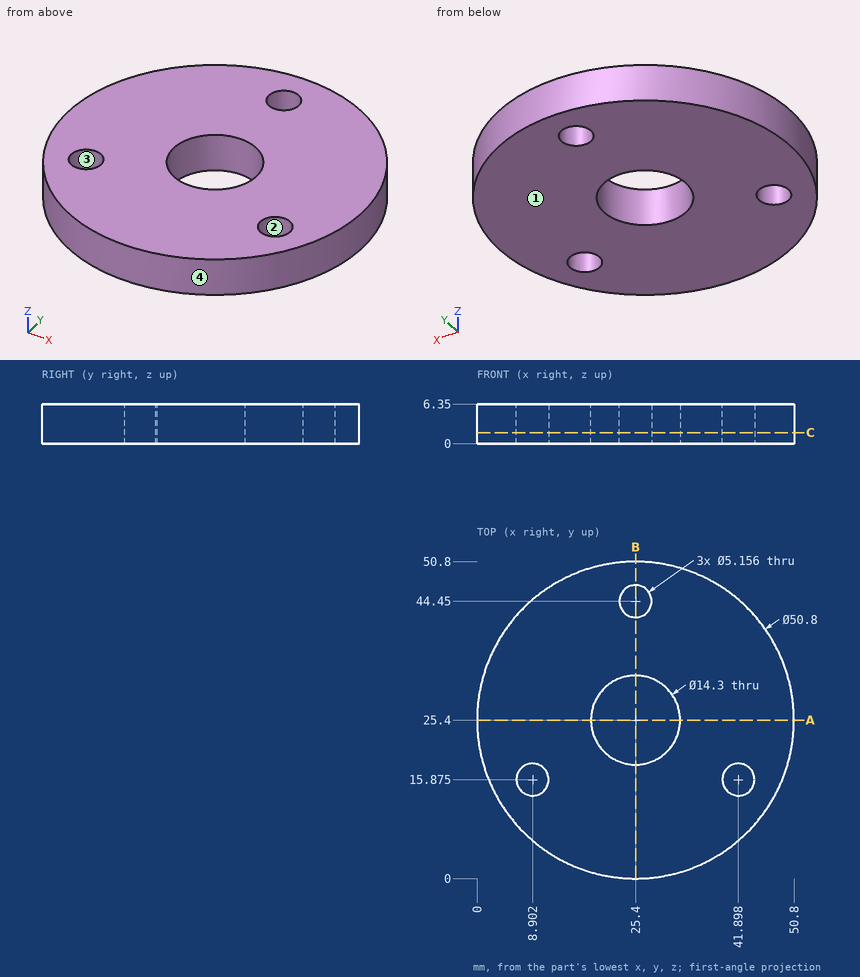
Answer from the drawing. Dimensions are ordinates in mm from the lowest x, y and z of the part. Give positions to 0.01 mm unless a question says otherwise; leave off trailing zeros. Order: outer loops, then holes, each group sorted by start corner. A loop starts at its lowest first (then second) coordinate and runs counter-clockwise, first axis right, second up.
(1) Find section B-B (x = 25.4). Give the vertices of the cut face in (y, z).
(2) Straight lines are drawn through the part: L1, parallel to Y at x = 25.4, z = 2.75; L2, parallel to X at y = 27, z = 2.25; L3, parallel to X at y = 20, z = 1. For each, find the intervals that lie inside material, in ascending order.
(3) Find section A-A (y = 25.4). Give the vertices of the cut face in (x, z), plus the area to 3 significant figures.
(4) Find section C-C (z = 1.75). Give the number of separate pieces and of enclosed holes in the cut face, plus the area to 3 significant figures.
(5) For a pull along X with two mould halves and no side action, classify the marked faces 1, 2, 3 and 4 as released by +X, released by -X, zero draft, split by the parting line, or undercut.
(6) Given pin 1 (1 mm diameter, centred on y = 33, z = 4, fed in from +X); pin 2 (18.5 mm diameter, centred on x = 25.4, y = 25.4, fed in from +Z); pin 3 (2 mm diameter, centred on x = 39, z = 1.5, fed in from -Y) (1 decimal), each flat-ended and moving along its own axis, determine where each tip first touches the part or whether it passes through.
Result sheet:
1. outline: (0, 0) - (18.25, 0) - (18.25, 6.35) - (0, 6.35) - close; (32.55, 0) - (41.87, 0) - (41.87, 6.35) - (32.55, 6.35) - close; (47.03, 0) - (50.8, 0) - (50.8, 6.35) - (47.03, 6.35) - close
2. L1: y = 0 to 18.25, 32.55 to 41.87, 47.03 to 50.8
2. L2: x = 0.05 to 18.43, 32.37 to 50.75
2. L3: x = 0.58 to 20.71, 30.09 to 50.22
3. outline: (0, 0) - (18.25, 0) - (18.25, 6.35) - (0, 6.35) - close; (32.55, 0) - (50.8, 0) - (50.8, 6.35) - (32.55, 6.35) - close
3. area: 232 mm2
4. separate pieces: 1
4. enclosed holes: 4
4. area: 1,800 mm2
5. face 1: zero draft
5. face 2: undercut
5. face 3: undercut
5. face 4: split by the parting line
6. pin 1: stops at x = 49.79
6. pin 2: stops at z = 6.35
6. pin 3: stops at y = 3.3
